The listing builds one solid part. Answer for the finished solid, in the listing's coordinates (mm). A direction names the side the tool comes from. Round coordinates to 2 decimals unless told otherwise and drop trailing zeros. Loops run counter-clockwise (first coordinate to the right, second up) from the corner with the lowest first, then second, coordinate; pieces in that order, holes last. Notation, with made-up numbers: (-9.5, 32) -> (-0.5, 32) arc R19 cw to (-0.5, 68) -> close; hole circle Ø10 at (-17.75, 80.25). An arc over 180 degrees is marked (long way). One line per question, with ' | ' between items.
from build123d import *

# Parameters (mm, degrees)
SKETCH1_R               = 70
BOSS_EXTRUDE1_DEPTH     = 26
SKETCH2_R               = 85
BOSS_EXTRUDE2_DEPTH     = 15
SKETCH3_R               = 60
BOSS_EXTRUDE3_DEPTH     = 40
CUT_EXTRUDE1_DEPTH      = 145.951716099
CUT_EXTRUDE1_DEPTH_BACK = 145.951716099
SKETCH4_R               = 25


with BuildPart() as part:
    # Sketch1 → Boss-Extrude1 (new body)
    with BuildSketch(Plane.XY):
        Circle(SKETCH1_R)
    extrude(amount=BOSS_EXTRUDE1_DEPTH)

    # Sketch2 → Boss-Extrude2 (add)
    with BuildSketch(Plane.XY.offset(26)):
        Circle(SKETCH2_R)
    extrude(amount=BOSS_EXTRUDE2_DEPTH)

    # Sketch3 → Boss-Extrude3 (add)
    with BuildSketch(Plane(origin=(0, 0, 0), x_dir=(-1, 0, 0), z_dir=(0, 0, -1))):
        Circle(SKETCH3_R)
    extrude(amount=BOSS_EXTRUDE3_DEPTH)

    # Sketch4 → Cut-Extrude1 (cut, two sides: drawn at the far end of the back side and taken through both)
    with BuildSketch(Plane.XY.offset(41).offset(-CUT_EXTRUDE1_DEPTH_BACK)):
        Circle(SKETCH4_R)
    extrude(amount=CUT_EXTRUDE1_DEPTH + CUT_EXTRUDE1_DEPTH_BACK, mode=Mode.SUBTRACT)


solid = part.part
Q1. Given pin 1 Ø6 at (x, z) = (-33.5, -18.5) entering from +Y; pin 2 Ø2 at (x, y) = (-51, 56) entering from -Z; pin 3 Ø10 at (y, z) = (58.5, -29.5) entering from -X, each flat-ended and moving along its own axis, determine where each tip first touches the part or whether it passes through.
Numbers:
pin 1: y = 51.67 | pin 2: z = 26 | pin 3: x = -27.16
Q2. A cutting plane is placed at C-C on z = -3. Give the vertices of the cut face in (x, y).
Numbers:
outline: circle Ø120 at (0, 0); hole circle Ø50 at (0, 0)
Q3. For faces 4 (the face through (59.94, 2.64, -19.72)), 5 (the face through (-26, 1, -40)), determine the directions among +Z, -Z, +X, -X, +Y, -Y from which every point of the face is accessible in a straight line to the end or side of a thin tool.
Numbers:
face 4: -Z | face 5: -Z, +X, -X, +Y, -Y
Q4. Find the intervals of material crossed by line 1 (Y direction, x = 0, z = 21); line 2 (X direction, y = -1.5, z = 19); line 3 (Y direction, x = 0, z = -23), in increasing order. Write a range as from..to.
Numbers:
line 1: -70..-25, 25..70 | line 2: -69.98..-24.95, 24.95..69.98 | line 3: -60..-25, 25..60
Q5. For a pull along Y with two mould halves and no side action, classify faces 1 (the face through (-55.55, -42.594, 12.818)), 2 (the face through (52, 31, 0)), 3 (the face through (23.846, 7.509, -0.067)) as pulls with the +Y half, pulls with the -Y half, needs draft (parallel to the pull), parting line crosses it, or undercut.
Numbers:
face 1: parting line crosses it | face 2: needs draft | face 3: undercut
Q6. A cutting plane is placed at A-A on x = 0. Give the vertices of the cut face in (y, z).
Numbers:
outline: (-85, 26) -> (-70, 26) -> (-70, 0) -> (-60, 0) -> (-60, -40) -> (-25, -40) -> (-25, 41) -> (-85, 41) -> close; (25, -40) -> (60, -40) -> (60, 0) -> (70, 0) -> (70, 26) -> (85, 26) -> (85, 41) -> (25, 41) -> close
Q7. A cutting plane is placed at D-D on y = 66. Give the vertices of the cut face in (x, z).
Numbers:
outline: (-53.56, 26) -> (-23.32, 26) -> (-23.32, 0) -> (23.32, 0) -> (23.32, 26) -> (53.56, 26) -> (53.56, 41) -> (-53.56, 41) -> close
